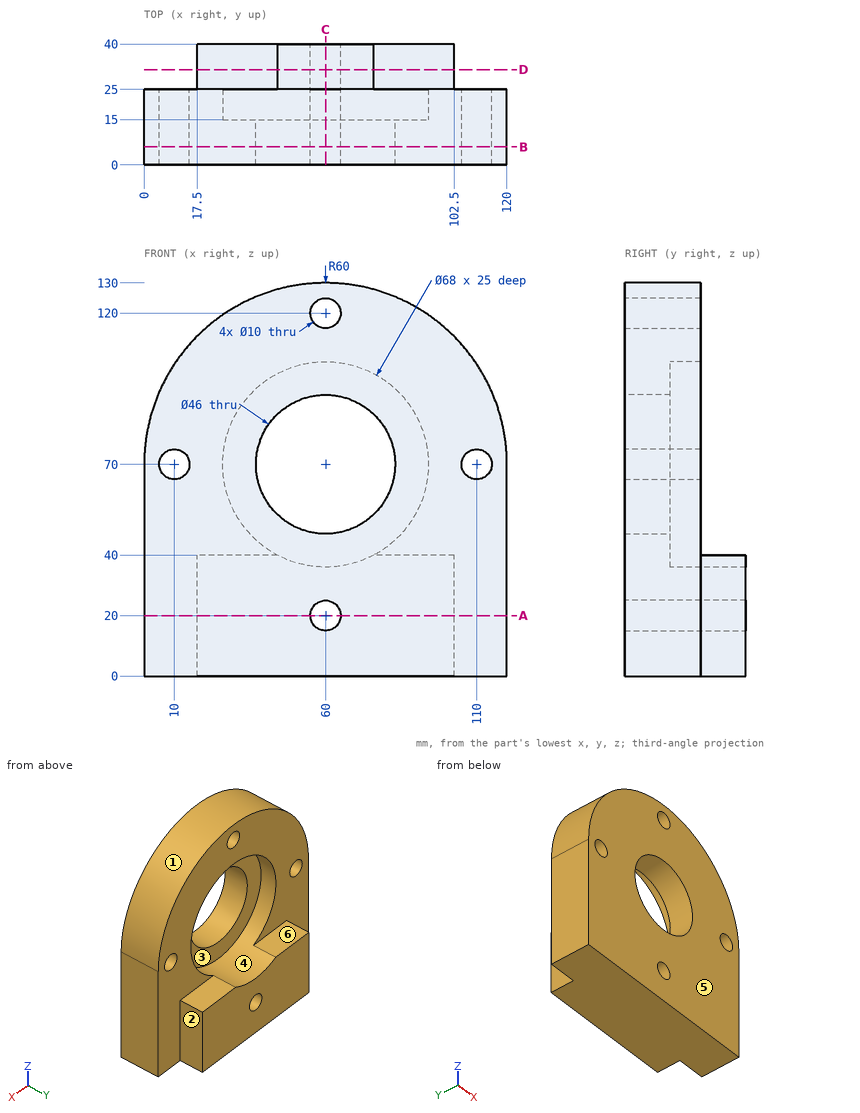
Geometry: see drawing. Coordinates: mm, zero at the bounding-box minimum. A direction names the side the tool comes from. Coordinates: 2 decimals unless noted, no trailing zeros. Order: outer loops, then holes, each group sorted by start corner. A loop starts at its lowest first (then second) coordinate and runs counter-clockwise, first axis right, second up. Notation, with made-up numbers: (29.5, 39) - (52.5, 39) arc R19 ccw to (52.5, 51) - close; hole circle Ø3 at (-31, -34.5). An arc over 180 degrees is marked (long way). Write each question's results on one line, items separated by ' | '.
1) Pull-direction query (Z, two-part tool) for the marked faces 1, 2 and 3; classes: pulls with the +Z half, pulls with the -Z half, needs draft (parallel to the pull), parting line crosses it, or undercut.
Results list:
face 1: pulls with the +Z half | face 2: needs draft | face 3: undercut
2) Section B-B, the plane y = 6. Return loops of the section in (x, z), plus the area to 3 significant figures.
Results list:
outline: (0, 0) - (120, 0) - (120, 70) arc R60 ccw to (0, 70) - close; hole circle Ø10 at (10, 70); hole circle Ø46 at (60, 70); hole circle Ø10 at (60, 20); hole circle Ø10 at (60, 120); hole circle Ø10 at (110, 70) | area: 12,100 mm^2
3) Section D-D, the plane y = 31.5. Return loops of the section in (x, z), plus the area to 3 significant figures.
Results list:
outline: (17.5, 0) - (102.5, 0) - (102.5, 40) - (76, 40) arc R34 cw to (44, 40) - (17.5, 40) - close; hole circle Ø10 at (60, 20) | area: 3,240 mm^2
4) Section A-A, the plane z = 20. Return loops of the section in (x, y).
Results list:
outline: (0, 0) - (55, 0) - (55, 40) - (17.5, 40) - (17.5, 25) - (0, 25) - close; (65, 0) - (120, 0) - (120, 25) - (102.5, 25) - (102.5, 40) - (65, 40) - close
5) Line query: line 1 (X direction, y = 7, z = 70); line 2 (X direction, y = 15.25, z = 70); line 3 (Y direction, x = 104, z = 22.5). Output: solid intervals per line, ascending. Write a range as from..to.
Results list:
line 1: 0..5, 15..37, 83..105, 115..120 | line 2: 0..5, 15..26, 94..105, 115..120 | line 3: 0..25
6) Pin query (flat end, axial travel): pin 1 (7.5 mm diameter, centred on y = 32.5, z = 20, fed in from -X); pin 2 (8 mm diameter, centred on x = 22.5, y = 33, fed in from +Z); pin 3 (5 mm diameter, centred on y = 17, z = 78.5, fed in from +X). Return the tip coordinate at first contact, or that it passes through.
Results list:
pin 1: x = 17.5 | pin 2: z = 40 | pin 3: x = 119.7
7) Section C-C, the plane x = 60. Return loops of the section in (y, z).
Results list:
outline: (0, 0) - (40, 0) - (40, 15) - (0, 15) - close; (0, 25) - (40, 25) - (40, 36) - (15, 36) - (15, 47) - (0, 47) - close; (0, 93) - (15, 93) - (15, 104) - (25, 104) - (25, 115) - (0, 115) - close; (0, 125) - (25, 125) - (25, 130) - (0, 130) - close
8) Set-up query: the marked faces 4, 5 and 6. Return all of +Z, -Z, +X, -X, +Y, -Y with unobstructed straight access to the full face (end or side cutting, diameter ignored); none if empty.
Results list:
face 4: +Y | face 5: +Z, -Z, +X, -X, -Y | face 6: +Z, +X, -X, +Y
